Can you work these out from the model? Positions are in its coordinate system, mm. Coordinates: 2 decimals unless noted, no trailing zeros. Order: outer loops, then holes, each group sorted by start corner. A loop starts at its lowest first (then second) coordinate and runs counter-clockwise, first axis right, second up. Notation, with made-up numbers: M 61,39 L 108,39 A18 ccw 108,52 Z; hole C 77,86.25 d11. An arc over 180 degrees is marked long. Answer as a JSON object with one key per item and string values.
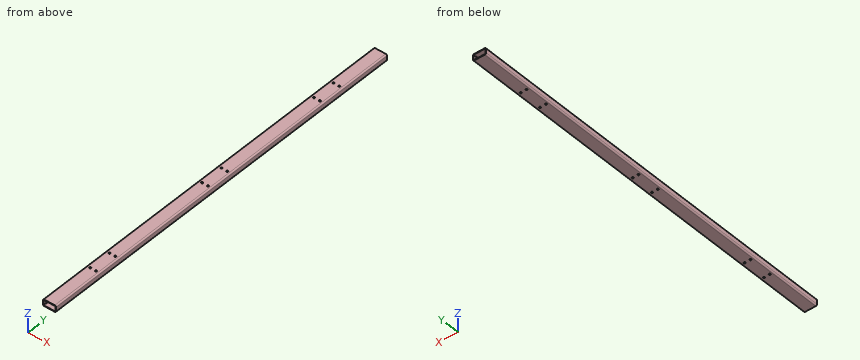
from build123d import *

# Parameters (mm, degrees)
F_40X20X2_1_DEPTH       = 1200
HOLE_WIZARD_5_2_5_2_1_D = 5.2
PATTERN_LINEAR_1_COUNT  = 3
PATTERN_LINEAR_1_PITCH  = 406


with BuildPart() as part:
    # Sketch1 → 矩型管 40X20X2(1) (new body)
    with BuildSketch(Plane.ZX):
        with BuildLine():
            Line((-6, -20), (6, -20))
            ThreePointArc((6, -20), (8.828427125, -18.828427125), (10, -16))
            Line((10, -16), (10, 16))
            ThreePointArc((10, 16), (8.828427125, 18.828427125), (6, 20))
            Line((6, 20), (-6, 20))
            ThreePointArc((-6, 20), (-8.828427125, 18.828427125), (-10, 16))
            Line((-10, 16), (-10, -16))
            ThreePointArc((-10, -16), (-8.828427125, -18.828427125), (-6, -20))
        make_face()
        with BuildLine():
            Line((-6, -18), (6, -18))
            ThreePointArc((6, -18), (7.414213562, -17.414213562), (8, -16))
            Line((8, -16), (8, 16))
            ThreePointArc((8, 16), (7.414213562, 17.414213562), (6, 18))
            Line((6, 18), (-6, 18))
            ThreePointArc((-6, 18), (-7.414213562, 17.414213562), (-8, 16))
            Line((-8, 16), (-8, -16))
            ThreePointArc((-8, -16), (-7.414213562, -17.414213562), (-6, -18))
        make_face(mode=Mode.SUBTRACT)
    extrude(amount=F_40X20X2_1_DEPTH)

    # Ø5.2 (5.2) 直径孔1 (through all)
    with Locations(Plane(origin=(0, 0, -10), x_dir=(-1, 0, 0), z_dir=(0, 0, -1))):
        with Locations((-9, 1040), (9, 1040), (9, 970), (-9, 970)):
            hole_wizard_5_2_5_2_1 = Hole(HOLE_WIZARD_5_2_5_2_1_D / 2)

    # 阵列(线性)1: Ø5.2 (5.2) 直径孔1 ×3
    with Locations(*[(0, -i * PATTERN_LINEAR_1_PITCH, 0) for i in range(1, PATTERN_LINEAR_1_COUNT)]):
        add(hole_wizard_5_2_5_2_1, mode=Mode.SUBTRACT)


solid = part.part
Item 1: I want a section at A-A, the plane z = -1.25. Write out the boundary of the cut face in (x, y), plus the area to 3 significant figures.
Answers follow:
{"outline": "M -20,0 L -18,0 L -18,1200 L -20,1200 Z; M 18,0 L 20,0 L 20,1200 L 18,1200 Z", "area": "4,800 mm^2"}
Item 2: I want a section at B-B, the plane y = 391. Write out the boundary of the cut face in (x, z).
Answers follow:
{"outline": "M -20,-6 A4 ccw -16,-10 L 16,-10 A4 ccw 20,-6 L 20,6 A4 ccw 16,10 L -16,10 A4 ccw -20,6 Z; hole M -18,-6 A2 ccw -16,-8 L 16,-8 A2 ccw 18,-6 L 18,6 A2 ccw 16,8 L -16,8 A2 ccw -18,6 Z"}
Item 3: Please list where these lines run through material, in increasing order: line 1 (X direction, y = 228, z = -9.5); line 2 (Z direction, x = 11.5, y = 1038); line 3 (X direction, y = 431.5, z = 0).
Answers follow:
{"line 1": "x = -17.94 to -11.6, -6.4 to 6.4, 11.6 to 17.94", "line 2": "z = -10 to -8, 8 to 10", "line 3": "x = -20 to -18, 18 to 20"}
